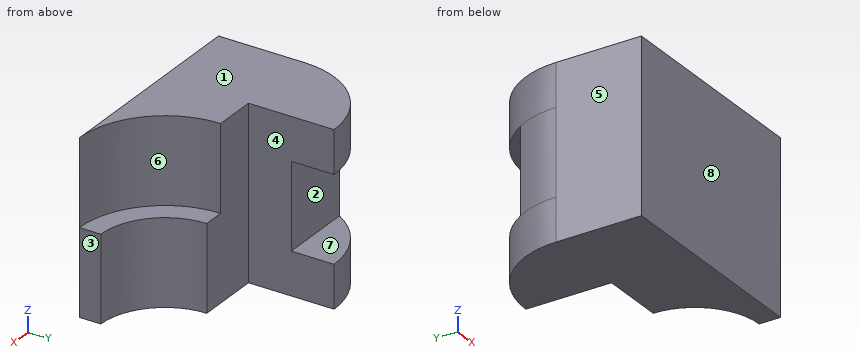
```python
from build123d import *

# Parameters (mm, degrees)
BASE_BLOCK_PROFILE_W      = 50
BASE_BLOCK_PROFILE_H      = 40
BASE_BLOCK_50X40X40_DEPTH = 20
CORNER_NOTCH_PROFILE_W    = 20
CORNER_NOTCH_PROFILE_H    = 20
CORNER_NOTCH_20X20_DEPTH  = 76.498344353
STEP_CUT_DEPTH            = 20
CONCAVE_ARC_CUT_DEPTH     = 20
ARC_GROOVE_CUT_DEPTH      = 76.498344353
TOP_SLOT_PROFILE_10X10_W  = 20
TOP_SLOT_PROFILE_10X10_H  = 23.40818189
TOP_SLOT_10X10_DEPTH      = 20
ROUNDED_TOP_CUT_DEPTH     = 20
RIDGE_BOSS_PROFILE_W      = 20
RIDGE_BOSS_PROFILE_H      = 20
RIDGE_BOSS_10_DEPTH       = 10
RIDGE_ROUND_CUT_DEPTH     = 20


with BuildPart() as part:
    # Base Block Profile → Base Block 50x40x40 (new, symmetric)
    with BuildSketch(Plane.XY):
        with Locations((25, 20)):
            Rectangle(BASE_BLOCK_PROFILE_W, BASE_BLOCK_PROFILE_H)
    extrude(amount=BASE_BLOCK_50X40X40_DEPTH, both=True)

    # Corner Notch Profile → Corner Notch 20x20 (cut, through all)
    with BuildSketch(Plane.XY.offset(20)):
        with Locations((40, 30)):
            Rectangle(CORNER_NOTCH_PROFILE_W, CORNER_NOTCH_PROFILE_H)
    extrude(amount=-CORNER_NOTCH_20X20_DEPTH, mode=Mode.SUBTRACT)

    # Step Cut Profile → Step Cut (cut)
    with BuildSketch(Plane.XY.offset(20)):
        with BuildLine():
            Line((50, 0), (50, 20))
            Line((50, 20), (30, 20))
            ThreePointArc((30, 20), (35.857864376, 5.857864376), (50, 0))
        make_face()
    extrude(amount=-STEP_CUT_DEPTH, mode=Mode.SUBTRACT)

    # Concave Arc Profile R30 → Concave Arc Cut (cut)
    with BuildSketch(Plane.XY):
        with BuildLine():
            Line((50, 5), (50, 20))
            Line((50, 20), (35, 20))
            ThreePointArc((35, 20), (39.393398282, 9.393398282), (50, 5))
        make_face()
    extrude(amount=-CONCAVE_ARC_CUT_DEPTH, mode=Mode.SUBTRACT)

    # Arc Groove Profile → Arc Groove Cut (cut, through all)
    with BuildSketch(Plane.XY.offset(20)):
        with BuildLine():
            Line((0, 40), (0, 20))
            ThreePointArc((0, 20), (5.857864376, 34.142135624), (20, 40))
            Line((20, 40), (0, 40))
        make_face()
    extrude(amount=-ARC_GROOVE_CUT_DEPTH, mode=Mode.SUBTRACT)

    # Top Slot Profile 10x10 → Top Slot 10x10 (cut)
    with BuildSketch(Plane.ZY):
        with Locations((0, 31.704090945)):
            Rectangle(TOP_SLOT_PROFILE_10X10_W, TOP_SLOT_PROFILE_10X10_H)
    extrude(amount=-TOP_SLOT_10X10_DEPTH, mode=Mode.SUBTRACT)

    # Rounded Top Profile → Rounded Top Cut (cut)
    with BuildSketch(Plane(origin=(0, 40, 0), x_dir=(1, 0, 0), z_dir=(0, 1, 0))):
        Polygon((20, 20), (20, 10), (20, -10), (20, -20), (30, -20), (30, 20), align=None)
    extrude(amount=-ROUNDED_TOP_CUT_DEPTH, mode=Mode.SUBTRACT)

    # Ridge Boss Profile → Ridge Boss 10 (add)
    with BuildSketch(Plane(origin=(0, 20, 0), x_dir=(1, 0, 0), z_dir=(0, 1, 0))):
        with Locations((10, 0)):
            Rectangle(RIDGE_BOSS_PROFILE_W, RIDGE_BOSS_PROFILE_H)
    extrude(amount=RIDGE_BOSS_10_DEPTH)

    # Ridge Round Profile → Ridge Round Cut (cut)
    with BuildSketch(Plane.XY.offset(10)):
        with BuildLine():
            Line((0, 30), (0, 20))
            ThreePointArc((0, 20), (0.681483474, 25.176380902), (2.679491924, 30))
            Line((2.679491924, 30), (0, 30))
        make_face()
    extrude(amount=-RIDGE_ROUND_CUT_DEPTH, mode=Mode.SUBTRACT)


solid = part.part
```
The model under review builds one solid part; all positions refer to its coordinate system, in mm. Face numbers are marked on the shaded views. A direction names the side the tool comes from. Round coordinates to 2 decimals unless told otherwise and drop trailing zeros. Order: outer loops, then holes, each group sorted by start corner. A loop starts at its lowest first (then second) coordinate and runs counter-clockwise, first axis right, second up. Notation, with made-up numbers: M 79.25,-10.5 L 132.25,-10.5 A25 cw 132.25,28.5 Z; hole C 2,26 d7. An arc over 180 degrees is marked long. Use a Markdown table: item, result.
1) Consider section B-B (y = 35). Write out the cut boundary in (x, z).
Report:
| item | result |
|---|---|
| outline | M 6.77,-20 L 20,-20 L 20,-10 L 6.77,-10 Z; M 6.77,10 L 20,10 L 20,20 L 6.77,20 Z |
2) Insertion check: pin 1 (4 mm diameter, centred on x = 6, z = 13, fed in from +Y); pin 2 (6 mm diameter, centred on y = 24.5, z = 2.5, fed in from -X); pin 3 (5 mm diameter, centred on x = 12.5, z = 3.5, fed in from +Y). Each pin has a flat end and moves straight along its axis. Give the tip position at first contact, or say it passes through.
Report:
| item | result |
|---|---|
| pin 1 | y = 36 |
| pin 2 | x = 0.06 |
| pin 3 | y = 30 |
3) Tool access review of the marked faces 4, 5, 6, 7 and 8: name each direction out of +Z, -Z, +X, -X, +Y, -Y from which nothing blocks a thin tool from reaching the whole face with its end or side.
Report:
| item | result |
|---|---|
| face 4 | +Z, -Z, +X, +Y |
| face 5 | +Z, -Z, -X, +Y, -Y |
| face 6 | +Z, +X, +Y |
| face 7 | +X, -X, +Y |
| face 8 | +Z, -Z, +X, -X, -Y |
4) Wall thickness on line 1 along Z through (x, y) = (35, 16); line 2 along Y through (x, z) = (7, -6); line 3 along Z through (x, y) = (11.5, 34): over which ranges is each line inside the solid? List them lowest first. Write a range as [from, to].
Report:
| item | result |
|---|---|
| line 1 | [-20, 0] |
| line 2 | [0, 30] |
| line 3 | [-20, -10], [10, 20] |
5) Draft analysis for pull direction Z (two halves, no side actions). For the marked faces 1, 2 and 3, state which applies: released by +Z, released by -Z, zero draft, split by the parting line, or undercut.
Report:
| item | result |
|---|---|
| face 1 | released by +Z |
| face 2 | undercut |
| face 3 | zero draft |
6) Consider section D-D (y = 12.5). Write out the cut boundary in (x, z), then the cut area to 3 significant figures.
Report:
| item | result |
|---|---|
| outline | M 0,-20 L 37.01,-20 L 37.01,0 L 31.46,0 L 31.46,20 L 0,20 Z |
| area | 1,370 mm^2 |
7) Consider section C-C (x = 10.5). Write out the cut boundary in (y, z), then the cut area to 3 significant figures.
Report:
| item | result |
|---|---|
| outline | M 0,-20 L 37.6,-20 L 37.6,-10 L 30,-10 L 30,10 L 37.6,10 L 37.6,20 L 0,20 Z |
| area | 1,350 mm^2 |
8) Consider section A-A (z = 3.5). Write out the cut boundary in (x, y), then the cut area to 3 significant figures.
Report:
| item | result |
|---|---|
| outline | M 0,0 L 50,0 A20 cw 30,20 L 20,20 L 20,30 L 2.68,30 A20 ccw 0,20 Z |
| area | 877 mm^2 |
